```python
from build123d import *

# Parameters (mm, degrees)
SKETCH1_W                  = 42
SKETCH1_H                  = 42
BOSS_EXTRUDE1_DEPTH        = 10
SKETCH2_R                  = 16.5
BOSS_EXTRUDE2_DEPTH        = 32
F_5_5_5_5_DIAMETER_HOLE1_D = 5.5
SKETCH7_R                  = 10
CUT_EXTRUDE1_DEPTH         = 52.439284598
CHAMFER1_SIZE              = 3


with BuildPart() as part:
    # Sketch1 → Boss-Extrude1 (new body)
    with BuildSketch(Plane(origin=(0, 0, 0), x_dir=(0, 0, -1), z_dir=(1, 0, 0))):
        Rectangle(SKETCH1_W, SKETCH1_H)
    extrude(amount=BOSS_EXTRUDE1_DEPTH)

    # Sketch2 → Boss-Extrude2 (add)
    with BuildSketch(Plane(origin=(10, 0, 0), x_dir=(0, 0, -1), z_dir=(1, 0, 0))):
        with Locations(Location((0, 0, 0), (0, 0, 180))):
            Circle(SKETCH2_R)
    extrude(amount=BOSS_EXTRUDE2_DEPTH)

    # Ø5.5 (5.5) Diameter Hole1 (through all)
    with Locations(Plane.ZY):
        with Locations((-15.202795796, 15.202795796), (15.202795796, 15.202795796), (15.202795796, -15.202795796), (-15.202795796, -15.202795796)):
            Hole(F_5_5_5_5_DIAMETER_HOLE1_D / 2)

    # Sketch7 → Cut-Extrude1 (cut, through all)
    with BuildSketch(Plane.ZY):
        Circle(SKETCH7_R)
    extrude(amount=-CUT_EXTRUDE1_DEPTH, mode=Mode.SUBTRACT)

    # Chamfer1
    chamfer1_edges = [part.edges().sort_by_distance(p)[0] for p in [
        (5, 21, -21),
        (5, -21, -21),
        (5, -21, 21),
        (5, 21, 21),
    ]]
    chamfer(chamfer1_edges, length=CHAMFER1_SIZE)


solid = part.part
```
Work out the finished part from the listing and answer in its coordinate system (mm). A direction names the side the tool comes from. Round coordinates to 2 decimals unless told otherwise and drop trailing zeros. Write each loop counter-clockwise with the first axis right and the second up, starting at its lowest first coordinate (ties: lowest second). Pieces come first, ordered by that corner, then holes. Notation, with made-up numbers: (-37, 8.25) -> (2, 8.25) arc R19 ccw to (2, 20.25) -> close; hole circle Ø9 at (-31, 83). An arc over 180 degrees is marked (long way). Write each question's results on one line, items separated by ' | '.
Q1. Flat-ended cylindrical pins translate along their axes: P1, Ø2, axis at y = 7, z = 5, coming from the +X side; P2, Ø8, axis at x = 21.5, z = -12.5, coming from the -Y side; P3, Ø2, axis at x = 19.5, y = -11.5, coming from the +Z side; P4, Ø1, axis at x = 13.5, y = 3.5, coming from the -Z side (3 decimals). Find the tip coordinate at first contact, or state that the pin passes through.
Data:
P1: through | P2: y = -14.14 | P3: z = 12.73 | P4: z = -16.225
Q2. Section C-C, the plane x = 11 is taken. Write down the section's boundary in (y, z).
Data:
outline: circle Ø33 at (0, 0); hole circle Ø20 at (0, 0)
Q3. Determine the mould class of faces 3 (the flat face through (5, 19, -20)), 4 (the flat face through (42, 11, 0)), 5 (the cylindrical face through (5.07, -12.884, -16.681)), 6 (the flat face through (5, -20, 19)) for opening direction Z: released by +Z, released by -Z, zero draft, split by the parting line, or undercut.
Data:
face 3: released by -Z | face 4: zero draft | face 5: undercut | face 6: released by +Z
Q4. Which of the six approach directions +Z, -Z, +X, -X, +Y, -Y give full straight-line access (tool end or side, diameter ignored) to faces 1 (the flat face through (5, 21, 0)), 2 (the flat face through (10, 14, 10))?
Data:
face 1: +Z, -Z, +X, -X, +Y | face 2: +X
Q5. Straight lines are drawn through the part: line 1 along Y through (x, z) = (6.5, 15); line 2 along Y through (x, z) = (7, -17.5); line 3 along Y through (x, z) = (5, -1.5). For each, find the intervals that lie inside material, in ascending order. Write a range as [from, to].
Data:
line 1: [-21, -17.95], [-12.46, 12.46], [17.95, 21] | line 2: [-21, -16.71], [-13.69, 13.69], [16.71, 21] | line 3: [-21, -9.89], [9.89, 21]
Q6. Section A-A, the plane y = 0 is taken. Write down the section's boundary in (x, z), then the cut area to 3 significant figures.
Data:
outline: (0, -21) -> (10, -21) -> (10, -16.5) -> (42, -16.5) -> (42, -10) -> (0, -10) -> close; (0, 10) -> (42, 10) -> (42, 16.5) -> (10, 16.5) -> (10, 21) -> (0, 21) -> close | area: 636 mm^2
